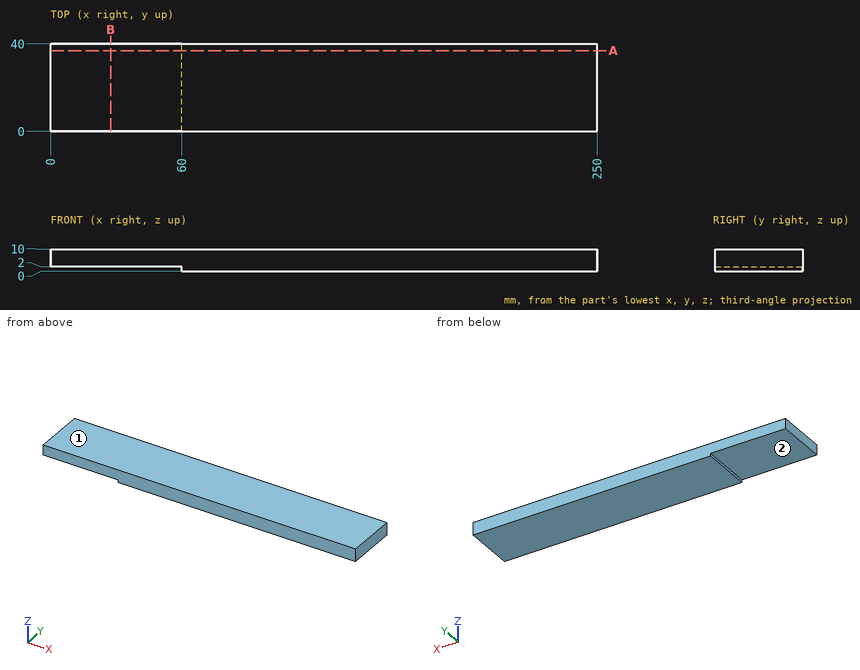
The figure shows three views and two pictorial views of one solid part (mm, origin at its lowest corner). Answer the questions. A direction names the side the tool comes from. Coordinates: 2 decimals unless noted, no trailing zeros. Write each loop counter-clockwise with the first axis right and the second up, starting at its lowest first coordinate (ties: lowest second). Pieces come first, ordered by that corner, then holes. Notation, with made-up numbers: (-12, 69.25) -> (26, 69.25) arc R12 ccw to (26, 75.25) -> close; hole circle Ø8 at (-31.5, 56.5). An arc over 180 degrees is marked (long way). Answer as a JSON object with one key per item and string values.
Q1. The part is cut by section B-B on x = 27.5. Give the vertices of the cut face in (y, z).
The answers:
{"outline": "(0, 2) -> (40, 2) -> (40, 10) -> (0, 10) -> close"}
Q2. Consider line 1 (Z direction, x = 22, y = 30.5); line 2 (X direction, y = 35, z = 1.25). Determine where each line is inside the solid, lowest interval first. Write a range as [from, to].
The answers:
{"line 1": "z = [2, 10]", "line 2": "x = [60, 250]"}
Q3. A flat-ended cylindrical pin translates along its axis: pin 1 Ø0.6 at (y, z) = (22, 1.5) entering from -X. Find the tip coordinate at first contact, or state that the pin passes through.
The answers:
{"pin 1": "stops at x = 60"}
Q4. The part is cut by section A-A on y = 37. Give the vertices of the cut face in (x, z), then the cut area to 3 significant figures.
The answers:
{"outline": "(0, 2) -> (60, 2) -> (60, 0) -> (250, 0) -> (250, 10) -> (0, 10) -> close", "area": "2,380 mm2"}
Q5. A tool of negligible diameter and unlimited length cuts with its end or side. For the marked faces 1 and 2, from which of +Z, -Z, +X, -X, +Y, -Y can it reach the whole face along a straight path? Write none if from no direction.
The answers:
{"face 1": "+Z, +X, -X, +Y, -Y", "face 2": "-Z, -X, +Y, -Y"}
